Geometry check sheet. Reference: drawing and pictorial views, mm from the part's lowest x, y, z. Give positions to 0.01 mm unless a question says otherwise; leave off trailing zeros. Order: outer loops, then holes, each group sorted by start corner. A loop starts at its lowest first (then second) coordinate and runs counter-clockwise, first axis right, second up. Notation, with made-up numbers: M 11.25,78.5 L 44.25,78.5 A21 cw 44.25,106.5 Z; hole C 15,85 d5. An arc over 180 degrees is marked long. Answer as CSV lines item,"result".
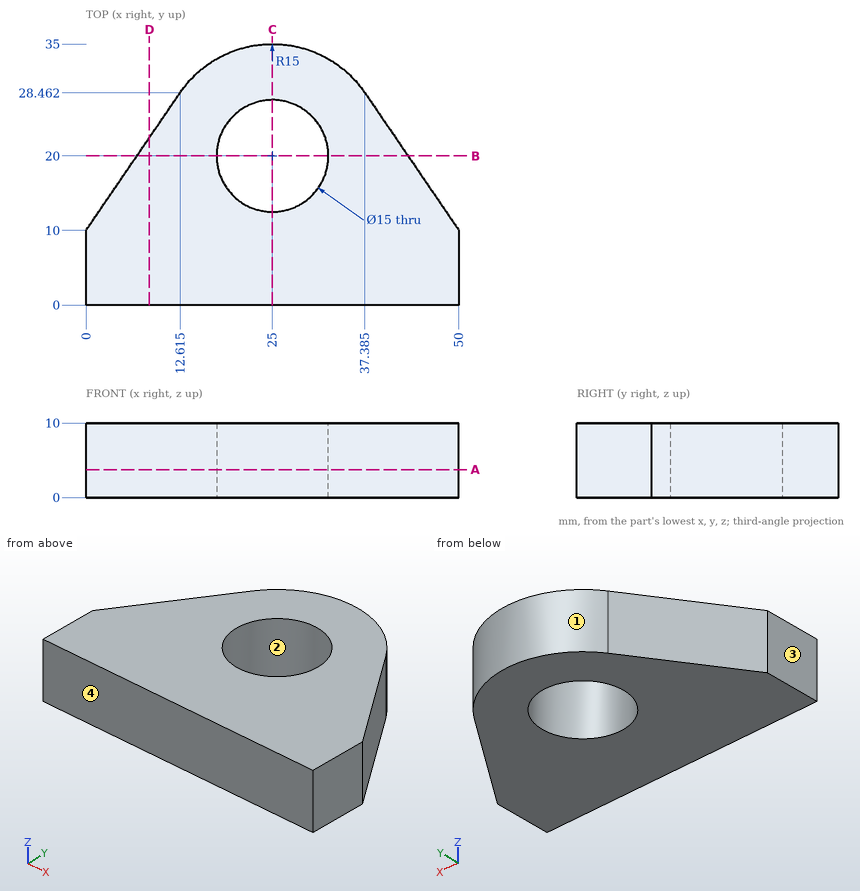
(1) Section check D-D on x = 8.5. Enter the section's corners in (y, z).
The answers:
outline,"M 0,0 L 22.44,0 L 22.44,10 L 0,10 Z"
(2) Section check C-C on x = 25. Enter the section's corners in (y, z), then the cut area to 3 significant figures.
The answers:
outline,"M 0,0 L 12.5,0 L 12.5,10 L 0,10 Z; M 27.5,0 L 35,0 L 35,10 L 27.5,10 Z"
area,"200 mm2"
(3) Draft check along Y on the marked faces 1, 2, 3 and 4. Enter one of: +Y half, -Y half, draft (parallel to the pull), parting line (faces both ways), or undercut.
The answers:
face 1,"+Y half"
face 2,"undercut"
face 3,"draft"
face 4,"-Y half"
(4) Section check B-B on y = 20. Enter the section's corners in (x, z).
The answers:
outline,"M 6.83,0 L 17.5,0 L 17.5,10 L 6.83,10 Z; M 32.5,0 L 43.17,0 L 43.17,10 L 32.5,10 Z"
(5) Section check A-A on z = 3.75. Enter the section's corners in (x, y) (1 decimal), then the cut area to 3 significant figures.
The answers:
outline,"M 0,0 L 50,0 L 50,10 L 37.4,28.5 A15 ccw 12.6,28.5 L 0,10 Z; hole C 25,20 d15"
area,"1,130 mm2"
(6) Material ranges on line 1 (Y direction, x = 25, z = 8); line 2 (X direction, y = 24, z = 2) (1 decimal); line 3 (X direction, y = 15, z = 7) (1 decimal), recorded low to high.
The answers:
line 1,"y = 0 to 12.5, 27.5 to 35"
line 2,"x = 9.6 to 18.7, 31.3 to 40.4"
line 3,"x = 3.4 to 19.4, 30.6 to 46.6"
(7) Gauge pin test, flat ends, axial feed: P1, Ø2, axis at x = 35, z = 1.5, coming from the +Y side; P2, Ø1, axis at x = 41.5, z = 3, coming from the +Y side; P3, Ø1.5, axis at y = 17.5, z = 2, coming from the -X side. Record the tip position at first contact, or that the pin passes through.
The answers:
P1,"stops at y = 32"
P2,"stops at y = 23.17"
P3,"stops at x = 4.61"
